```python
from build123d import *

# Parameters (mm, degrees)
EXTRUDE_1_DEPTH    = 472.5
HOLE_WIZARD_M4_1_D = 4.8
CHAMFER_1_SIZE     = 10
HOLE_WIZARD_M5_1_D = 4.2


with BuildPart() as part:
    # 草图1 → 凸台-拉伸1 (new, symmetric)
    with BuildSketch(Plane.XY):
        Polygon((0, 0), (60, 0), (60, 60), (57, 60), (57, 3), (0, 3), align=None)
    extrude(amount=EXTRUDE_1_DEPTH, both=True)

    # M4 间隙孔1 (through all)
    with Locations(Plane(origin=(0, 3, 0), x_dir=(1, 0, 0), z_dir=(0, 1, 0))):
        with Locations((47, 0), (47, 232.25), (47, 464.5), (47, -464.5), (47, -232.25), (47, 449.5), (47, -449.5)):
            Hole(HOLE_WIZARD_M4_1_D / 2)

    # 倒角1
    chamfer_1_edges = [part.edges().sort_by_distance(p)[0] for p in [
        (58.5, 60, 472.5),
        (0, 1.5, 472.5),
        (58.5, 60, -472.5),
        (0, 1.5, -472.5),
    ]]
    chamfer(chamfer_1_edges, length=CHAMFER_1_SIZE)

    # M5 螺纹孔1 (through all)
    with Locations(Plane(origin=(0, 3, 0), x_dir=(1, 0, 0), z_dir=(0, 1, 0))):
        with Locations((9.75, 373.7), (39.75, 373.7), (24.75, 358.7), (9.75, 358.7), (39.75, 358.7), (24.75, 373.7)):
            Hole(HOLE_WIZARD_M5_1_D / 2)


solid = part.part
```
Check sheet for the modelled part. Datum: model origin and axes. Units: mm. A direction names the side the tool comes from. Give positions to 0.01 mm unless a question says otherwise; leave off trailing zeros. Write each loop counter-clockwise with the first axis right and the second up, starting at its lowest first coordinate (ties: lowest second). Pieces come first, ordered by that corner, then holes.
Item 1: Cross-section at A-A (z = -48.5). Enter the section's corners in (x, y), and give its area (3 significant figures).
Item 2: Gauge pin test, flat ends, axial feed: pin 1 (5 mm diameter, centred on x = 26, z = 234.5, fed in from +Y); pin 2 (12 mm diameter, centred on y = 24, z = -257, fed in from -X). Record the tip position at first contact, or that the pin passes through.
Item 3: Scan lines: L1, parallel to X at y = 1.6, z = -358.7; L2, parallel to X at y = 1, z = -373; L3, parallel to Z at x = 39, y = 2. Record each from-to range of solid material in increasing order.
Item 4: Access from +Z, -Z, +X, -X, +Y, -Y to the whole of each face (thin tool, end or side, straight path). Record for faces 1 (the face through (30, 0, 7)), 2 (the face through (29, 3, 7)).
Report:
1. outline: (0, 0) - (60, 0) - (60, 60) - (57, 60) - (57, 3) - (0, 3) - close
1. area: 351 mm2
2. pin 1: stops at y = 3
2. pin 2: stops at x = 57
3. L1: x = 0 to 7.65, 11.85 to 22.65, 26.85 to 37.65, 41.85 to 60
3. L2: x = 0 to 7.77, 11.73 to 22.77, 26.73 to 37.77, 41.73 to 60
3. L3: z = -472.5 to -375.66, -371.74 to -360.66, -356.74 to 472.5
4. face 1: +Z, -Z, +X, -X, -Y
4. face 2: +Z, -Z, -X, +Y
